from build123d import *

# Parameters (mm, degrees)
SKETCH_1_W          = 24
SKETCH_1_H          = 15
SKETCH_1_W_2        = 15
SKETCH_1_H_2        = 10
SKETCH_3_R          = 1.75
CUT_EXTRUDE_1_DEPTH = 5
SKETCH_4_R          = 1.75
CUT_EXTRUDE_2_DEPTH = 5


with BuildPart() as part:
    # 扫描1: sweep along a path in 草图2
    with BuildLine(Plane(origin=(0, 0, 0), x_dir=(0, 0, -1), z_dir=(1, 0, 0))) as sweep_1_path:
        Line((0, 0), (120, 0))
        ThreePointArc((120, 0), (148, 28), (120, 56))
        Line((120, 56), (-220, 56))
    # 草图1 → 扫描1 (sweep)
    with BuildSketch(Plane.XY):
        Rectangle(SKETCH_1_W, SKETCH_1_H)
        Rectangle(SKETCH_1_W_2, SKETCH_1_H_2, mode=Mode.SUBTRACT)
    sweep(path=sweep_1_path.line)

    # 草图3 → 切除-拉伸1 (cut)
    with BuildSketch(Plane(origin=(0, 63.5, 0), x_dir=(1, 0, 0), z_dir=(0, 1, 0))):
        with Locations(Location((0, -214.5, 0), (0, 0, 180))):
            Circle(SKETCH_3_R)
        with Locations(Location((0, -205.5, 0), (0, 0, 180))):
            Circle(SKETCH_3_R)
    extrude(amount=-CUT_EXTRUDE_1_DEPTH, mode=Mode.SUBTRACT)

    # 草图4 → 切除-拉伸2 (cut)
    with BuildSketch(Plane.XZ.offset(7.5)):
        with Locations((0, -5.5)):
            Circle(SKETCH_4_R)
        with Locations((0, -14.5)):
            Circle(SKETCH_4_R)
    extrude(amount=-CUT_EXTRUDE_2_DEPTH, mode=Mode.SUBTRACT)


solid = part.part
Can you work these out from the model? Positions are in its coordinate system, mm. A direction names the side the tool comes from. Coordinates: 2 decimals unless noted, no trailing zeros. Loops run counter-clockwise (first coordinate to the right, second up) from the corner with the lowest first, then second, coordinate; pieces in that order, holes last. Notation, with made-up numbers: (84, 48) - (115, 48) arc R23 ccw to (115, 66) - close; hole circle Ø11 at (87.5, 14.5). An arc over 180 degrees is marked (long way). Answer as a JSON object with one key per item and string values. Group by question number.
Item 1: If we section it at B-B (y = 28): List the corners of the cut face in (x, z) for me, plus the area to 3 significant figures.
Item 2: If we section it at D-D (y = -1): List the corners of the cut face in (x, z) for me.
Item 3: If we mould it in two halves opening along X, with no side actions, what happens to faces 5 (the face through (7.5, 53, -9)), 6 (the face through (-12, 49, -10)), 7 (the face through (0, 7, 0))? For each: released by +X, released by -X, zero draft, split by the parting line, or undercut.
Item 4: If I drill on L1, parallel to Y at x = 2.25, z = -9; L2, parallel to X at y = 61.6, z = 214.5; L3, parallel to Y at x = 3.5, z = 103.5, over which ranges is the centre line in solid material (lowest first)? Write a range as from..to.
Item 5: On a 3-axis mill with a long thin cutter (end or side, diameter ignored), from which of +Z, -Z, +X, -X, +Y, -Y can I reach the whole of each face in a straight line? I mean faces 1 (the face through (0.17, 27.22, -155.49)), 2 (the face through (0, -5, -61)), 3 (the face through (0, 48.5, 52)), 4 (the face through (-7.5, 55, -9)). Say none if no direction works.
Item 6: If we section it at C-C (z = 125): List the corners of the cut face in (x, y) for me.
Item 7: If we section it at A-A (z = -26): List the corners of the cut face in (x, y) for me, plus the area to 3 significant figures.
Item 8: For pin 1 (5 mm diameter, centred on x = 1.5, z = 48.5, fed in from -Y); pin 2 (3 mm diameter, centred on x = -8.5, y = 29.5, fed in from -Z); pin 3 (1 mm diameter, centred on x = 4.5, y = 39, fed in from -Z); pin 4 (20 mm diameter, centred on y = 35, z = 1, fed in from -X), each with a flat end and sliding along its axis, tell me the tip position at first contact or that it passes through.
Returned:
{
 "1": {"outline": "(-12, -155.5) - (12, -155.5) - (12, -140.5) - (-12, -140.5) - close; hole (-7.5, -153) - (7.5, -153) - (7.5, -143) - (-7.5, -143) - close", "area": "210 mm²"},
 "2": {"outline": "(-12, -140.48) - (12, -140.48) - (12, 0) - (7.5, 0) - (7.5, -135.75) - (-7.5, -135.75) - (-7.5, 0) - (-12, 0) - close"},
 "3": {"face 5": "undercut", "face 6": "released by -X", "face 7": "zero draft"},
 "4": {"L1": "y = -7.5..-5, 5..7.5, 48.5..51, 61..63.5", "L2": "x = -12..-1.75, 1.75..12", "L3": "y = 48.5..51, 61..63.5"},
 "5": {"face 1": "-Z, +X, -X", "face 2": "+Z", "face 3": "+Z, +X, -X", "face 4": "none"},
 "6": {"outline": "(-12, 48.5) - (12, 48.5) - (12, 63.5) - (-12, 63.5) - close; hole (-7.5, 51) - (7.5, 51) - (7.5, 61) - (-7.5, 61) - close"},
 "7": {"outline": "(-12, -7.5) - (12, -7.5) - (12, 7.5) - (-12, 7.5) - close; (-12, 48.5) - (12, 48.5) - (12, 63.5) - (-12, 63.5) - close; hole (-7.5, -5) - (7.5, -5) - (7.5, 5) - (-7.5, 5) - close; hole (-7.5, 51) - (7.5, 51) - (7.5, 61) - (-7.5, 61) - close", "area": "420 mm²"},
 "8": {"pin 1": "stops at y = 48.5", "pin 2": "stops at z = -155.5", "pin 3": "stops at z = -153.91", "pin 4": "passes through"}
}
